from build123d import *

# Parameters (mm, degrees)
JAW_BODY_12MM_DEPTH       = 6
END_BOSS_SKETCH_R         = 6
END_BOSS_DEPTH            = 12
CUT_4_8_SKETCH_R          = 2.4
CUT_4_8_X_6_DEPTH         = 6
TAPPED_HOLE_M8X1_25_D     = 8
TAPPED_HOLE_M8X1_25_DEPTH = 19.75
TAPPED_HOLE_M8X1_25_TIP   = 2.403442476
TAPPED_HOLE_M3X0_5_D      = 3
TAPPED_HOLE_M3X0_5_DEPTH  = 8
TAPPED_HOLE_M3X0_5_TIP    = 0.901290929


with BuildPart() as part:
    # Jaw Profile Sketch → Jaw Body 12mm (new, symmetric)
    with BuildSketch(Plane.XY):
        Polygon((0, 0), (5, 0), (12, -30), (12, -74), (0, -74), align=None)
    extrude(amount=JAW_BODY_12MM_DEPTH, both=True)

    # End Boss Sketch → End Boss (add)
    with BuildSketch(Plane.ZY):
        with Locations((0, -74)):
            Circle(END_BOSS_SKETCH_R)
    extrude(amount=-END_BOSS_DEPTH)

    # Cut Ø4.8 Sketch → Cut Ø4.8 x 6 (cut)
    with BuildSketch(Plane.ZY):
        with Locations((0, -74)):
            Circle(CUT_4_8_SKETCH_R)
    extrude(amount=-CUT_4_8_X_6_DEPTH, mode=Mode.SUBTRACT)

    # Tapped Hole M8x1.25
    with Locations(Plane(origin=(12, -39, 0), x_dir=(0, 1, 0), z_dir=(1, 0, 0))):
        with Locations((0, 0)):
            Hole(TAPPED_HOLE_M8X1_25_D / 2, depth=TAPPED_HOLE_M8X1_25_DEPTH)
            with Locations((0, 0, -(TAPPED_HOLE_M8X1_25_DEPTH + TAPPED_HOLE_M8X1_25_TIP / 2))):  # 118° drill point
                Cone(0, TAPPED_HOLE_M8X1_25_D / 2, TAPPED_HOLE_M8X1_25_TIP, mode=Mode.SUBTRACT)

    # Tapped Hole M3x0.5
    with Locations(Plane(origin=(12, -57, 0), x_dir=(0, 1, 0), z_dir=(1, 0, 0))):
        with Locations((0, 0)):
            Hole(TAPPED_HOLE_M3X0_5_D / 2, depth=TAPPED_HOLE_M3X0_5_DEPTH)
            with Locations((0, 0, -(TAPPED_HOLE_M3X0_5_DEPTH + TAPPED_HOLE_M3X0_5_TIP / 2))):  # 118° drill point
                Cone(0, TAPPED_HOLE_M3X0_5_D / 2, TAPPED_HOLE_M3X0_5_TIP, mode=Mode.SUBTRACT)


solid = part.part
Model file for the job. Use its own axes, mm. A direction names the side the tool comes from. Give positions to 0.01 mm unless a question says otherwise; leave off trailing zeros. Order: outer loops, then holes, each group sorted by start corner. A loop starts at its lowest first (then second) coordinate and runs counter-clockwise, first axis right, second up. Notation, with made-up numbers: (35, 37) - (41, 37) arc R23 cw to (41, 70) - close; hole circle Ø3 at (-27, 16). An arc over 180 degrees is marked (long way). Return JSON: item names as keys, results as strings.
1) Cut at A-A, the plane y = -39. Give the cut face in (x, z), plus the area to 3 significant figures.
Geometry says:
{"outline": "(0, -6) - (12, -6) - (12, -4) - (0, -4) - close; (0, 4) - (12, 4) - (12, 6) - (0, 6) - close", "area": "48.0 mm²"}
2) Cut at D-D, the plane z = 5.25. Give the cut face in (x, y).
Geometry says:
{"outline": "(0, -76.9) - (12, -76.9) - (12, -30) - (5, 0) - (0, 0) - close"}
3) Pull direction Z, two halves, no side cores. Call faces 4 (the cylindrical face through (6, -80, 0)), 5 (the flat face through (6, -36, 6)), 6 (the cylindrical face through (2.96, -71.62, -0.31)): pulls with the +Z half, pulls with the -Z half, needs draft (parallel to the pull), parting line crosses it, or undercut.
Geometry says:
{"face 4": "parting line crosses it", "face 5": "pulls with the +Z half", "face 6": "undercut"}
4) Cut at C-C, the plane x = 9. Give the cut face in (y, z), plus the area to 4 significant figures.
Geometry says:
{"outline": "(-74, -6) - (-17.14, -6) - (-17.14, 6) - (-74, 6) arc R6 ccw to start; hole circle Ø3 at (-57, 0); hole circle Ø8 at (-39, 0)", "area": "681.5 mm²"}
5) Cut at B-B, the plane y = -72.5. Give the cut face in (x, z).
Geometry says:
{"outline": "(0, -6) - (12, -6) - (12, 6) - (0, 6) - (0, 1.87) - (6, 1.87) - (6, -1.87) - (0, -1.87) - close"}
6) 3-axis set-ups, long thin cutter, end or side, ignore diameter. For faces 1 (the cylindrical face through (7.94, -58.43, 0.45)), 2 (the flat face through (6, -74, 0)), 3 (the flat face through (2, 0, 0)): which of +Z, -Z, +X, -X, +Y, -Y reach the whole face in a straight line?
Geometry says:
{"face 1": "+X", "face 2": "-X", "face 3": "+Z, -Z, +X, -X, +Y"}
7) Flat gauge pins, fed straight in: P1, Ø1.5, axis at x = 9.5, z = -1, coming from the -Y side; P2, Ø3, axis at x = 9, z = -4.5, coming from the -Y side; P3, Ø3, axis at y = -74, z = 0, coming from the -X side. Where does each tip first touch, or does it go through?
Geometry says:
{"P1": "y = -79.99", "P2": "y = -79.2", "P3": "x = 6"}
8) Probe line 1 (Z direction, x = 3, y = -39); line 2 (Z direction, x = 7, y = -36); line 3 (X direction, y = -19.5, z = 0). List the from-to ranges inside material, lowest first. Write a range as from..to.
Geometry says:
{"line 1": "-6..-4, 4..6", "line 2": "-6..-2.65, 2.65..6", "line 3": "0..9.55"}
